Design review of the part built by this model. Coordinates are the model's own, in mm. Coordinates: 2 decimals unless noted, no trailing zeros. Order: outer loops, then holes, each group sorted by start corner. A loop starts at its lowest first (then second) coordinate and runs counter-clockwise, first axis right, second up. Notation, with made-up numbers: M -34,-17 L -29,-17 A35 cw -29,19 Z; hole C 34,59 d9. An arc over 180 degrees is marked long. Answer in a Markdown table with one row per item.
from build123d import *

# Parameters (mm, degrees)
SKETCH1_W           = 92
SKETCH1_H           = 92
BOSS_EXTRUDE1_DEPTH = 25
SKETCH2_R           = 40
CUT_EXTRUDE1_DEPTH  = 25
SKETCH3_R           = 2
CUT_EXTRUDE2_DEPTH  = 30


with BuildPart() as part:
    # Sketch1 → Boss-Extrude1 (new body)
    with BuildSketch(Plane.XY):
        with Locations((-46, 46)):
            Rectangle(SKETCH1_W, SKETCH1_H)
    extrude(amount=BOSS_EXTRUDE1_DEPTH)

    # Sketch2 → Cut-Extrude1 (cut)
    with BuildSketch(Plane.XY.offset(25)):
        with Locations((-45, 45)):
            Circle(SKETCH2_R)
    extrude(amount=-CUT_EXTRUDE1_DEPTH, mode=Mode.SUBTRACT)

    # Sketch3 → Cut-Extrude2 (cut)
    with BuildSketch(Plane.XY.offset(25)):
        with Locations((-4.75, 87.599810623)):
            Circle(SKETCH3_R)
        with Locations((-87.25, 87.599810623)):
            Circle(SKETCH3_R)
        with Locations((-87.25, 4.400189377)):
            Circle(SKETCH3_R)
        with Locations((-4.75, 4.400189377)):
            Circle(SKETCH3_R)
    extrude(amount=-CUT_EXTRUDE2_DEPTH, mode=Mode.SUBTRACT)


solid = part.part
(1) Insertion check: pin 1 Ø3.5 at (x, y) = (-4.75, 87.6) entering from +Z. The pin has a flat end and moves straight along its axis. Give the tip position at first contact, or say it passes through.
Return value:
| item | result |
|---|---|
| pin 1 | passes through |
(2) For line 1 along Y through (x, z) = (-4.75, 17); line 2 along Y through (x, z) = (-45, 6); line 3 along Y through (x, z) = (-55.5, 8), list the stretches that pass through material, from the lowest coordinate up. Write a range as from..to.
Return value:
| item | result |
|---|---|
| line 1 | y = 0..2.4, 6.4..85.6, 89.6..92 |
| line 2 | y = 0..5, 85..92 |
| line 3 | y = 0..6.4, 83.6..92 |
(3) Draft analysis for pull direction X (two halves, no side actions). For faces 1 (the cylindrical face through (-85.34, 5, 12.68)), 2 (the cylindrical face through (-53.67, 5.95, 12.68)), 3 (the flat face through (-47, 0, 12)), 4 (the flat face through (0, 45, 12)), state which applies: pulls with the +X half, pulls with the -X half, needs draft (parallel to the pull), parting line crosses it, or undercut.
Return value:
| item | result |
|---|---|
| face 1 | undercut |
| face 2 | undercut |
| face 3 | needs draft |
| face 4 | pulls with the +X half |
(4) Add section C-C, the plane z = 16.25. Give the boundary of the cut face in (x, y), and give its area (3 significant figures).
Return value:
| item | result |
|---|---|
| outline | M -92,0 L 0,0 L 0,92 L -92,92 Z; hole C -87.25,4.4 d4; hole C -87.25,87.6 d4; hole C -45,45 d80; hole C -4.75,4.4 d4; hole C -4.75,87.6 d4 |
| area | 3,390 mm2 |
(5) Add section A-A, the plane y = 45. Give the boundary of the cut face in (x, z).
Return value:
| item | result |
|---|---|
| outline | M -92,0 L -85,0 L -85,25 L -92,25 Z; M -5,0 L 0,0 L 0,25 L -5,25 Z |
(6) Add section B-B, the plane x = -45. Give the boundary of the cut face in (y, z), and give its area (3 significant figures).
Return value:
| item | result |
|---|---|
| outline | M 0,0 L 5,0 L 5,25 L 0,25 Z; M 85,0 L 92,0 L 92,25 L 85,25 Z |
| area | 300 mm2 |
